Could you check a few things on this drawing? It's one solid part, dimensions in mm from its lowest x, y, z. Give positions to 0.01 mm unless a question says otherwise; leave off trailing zeros. Order: outer loops, then holes, each group sorted by start corner. A loop starts at its lowest first (then second) coordinate and runs counter-clockwise, first axis right, second up. Notation, with made-up numbers: (31.5, 41) - (76.5, 41) arc R12 ccw to (76.5, 57) - close; hole circle Ø7 at (-14.75, 83.25). An arc over 180 degrees is marked (long way). Return JSON: item names as keys, results as strings.
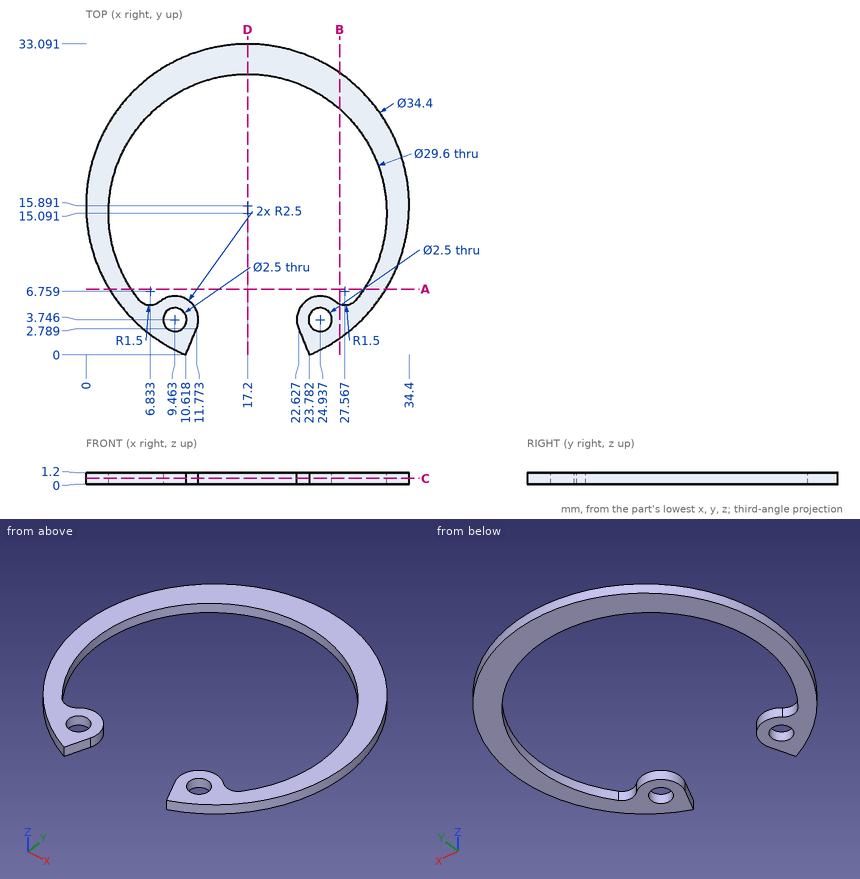
1. If I drill on L1, parallel to X at y = 6, z = 1.1 (1 decimal); L2, parallel to Y at x = 10, z = 0.15 (1 decimal); L3, parallel to Y at x = 27, z = 0.3 (1 decimal), over which ranges is the centre line in solid material (lowest first)? Write a range as [from, to].
Checks:
{"L1": "[3.1, 5.5], [8.4, 10.5], [23.9, 26], [28.9, 31.3]", "L2": "[0.3, 2.6], [4.9, 6.2], [28, 31.5]", "L3": "[1.8, 5.4], [26.2, 30]"}
2. Suppose I cut it at C-C (z = 0.6). State how many separate pieces and enclosed holes the cut face has, plus the area to 3 significant figures.
Checks:
{"separate pieces": "1", "enclosed holes": "2", "area": "242 mm^2"}
3. Suppose I cut it at D-D (x = 17.2). List the corners of the cut face in (y, z) for me.
Checks:
{"outline": "(29.89, 0) - (33.09, 0) - (33.09, 1.2) - (29.89, 1.2) - close"}
4. Suppose I cut it at B-B (x = 27). List the corners of the cut face in (y, z) for me (1 decimal).
Checks:
{"outline": "(1.8, 0) - (5.4, 0) - (5.4, 1.2) - (1.8, 1.2) - close; (26.2, 0) - (30, 0) - (30, 1.2) - (26.2, 1.2) - close"}
5. Suppose I cut it at A-A (y = 7). List the corners of the cut face in (x, z) for me.
Checks:
{"outline": "(2.48, 0) - (4.81, 0) - (4.81, 1.2) - (2.48, 1.2) - close; (29.59, 0) - (31.92, 0) - (31.92, 1.2) - (29.59, 1.2) - close"}
